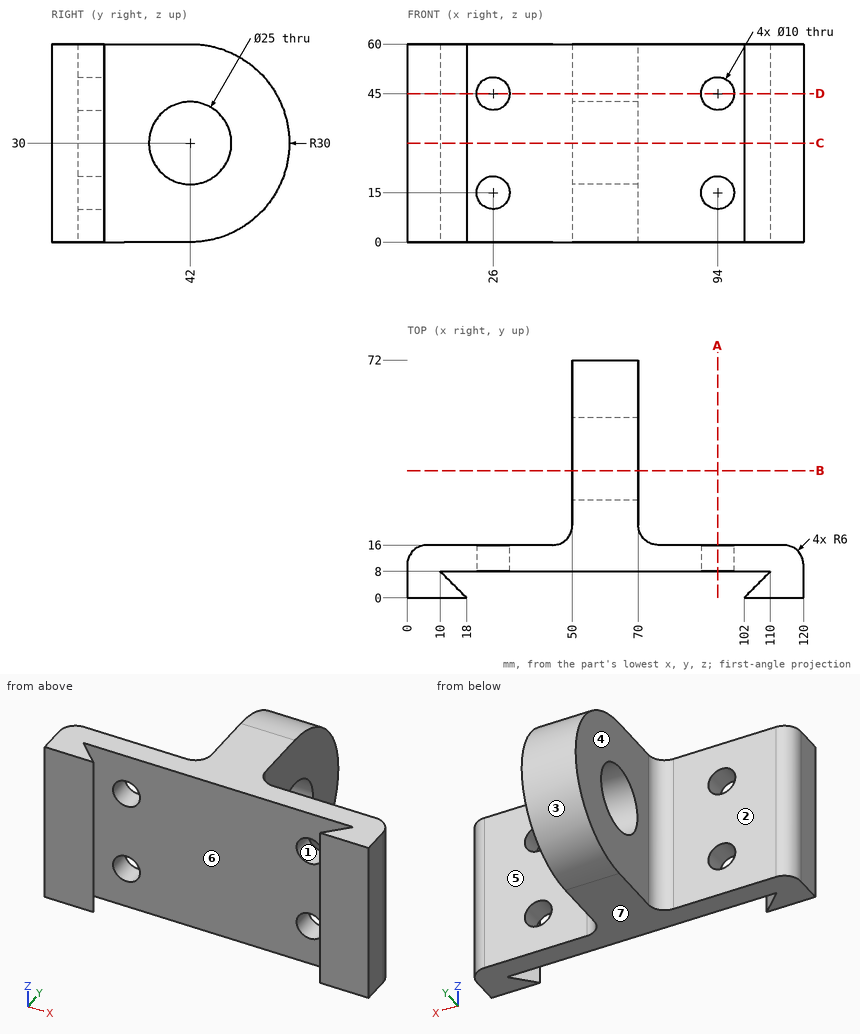
Drawing for the job (mm, zero at the part's lowest x, y, z). A direction names the side the tool comes from. Round coordinates to 2 decimals unless told otherwise and drop trailing zeros. Write each loop counter-clockwise with the first axis right and the second up, starting at its lowest first coordinate (ties: lowest second). Pieces come first, ordered by that corner, then holes. Notation, with made-up numbers: M 32.25,-36.75 L 65.25,-36.75 A8 ccw 65.25,-25.75 Z; hole C -37,3 d2. An arc over 180 degrees is marked long. Put each result on its own line as item: value.
Item 1: Cut at B-B (y = 38.5). List the corners of the cut face in (x, z), and give its area (3 significant figures).
Responses:
outline: M 50,0 L 70,0 L 70,18 L 50,18 Z; M 50,42 L 70,42 L 70,60 L 50,60 Z
area: 720 mm²
Item 2: Cut at C-C (z = 30). List the corners of the cut face in (x, y), and give its area (3 significant figures).
Responses:
outline: M 0,0 L 18,0 L 10,8 L 110,8 L 102,0 L 120,0 L 120,10 A6 ccw 114,16 L 76,16 A6 cw 70,22 L 70,29.5 L 50,29.5 L 50,22 A6 cw 44,16 L 6,16 A6 ccw 0,10 Z; M 50,54.5 L 70,54.5 L 70,72 L 50,72 Z
area: 1,800 mm²
Item 3: Tool access for the marked faces 4, 5, 6 and 7: list every direction of +Z, -Z, +X, -X, +Y, -Y with a clear straight run to the whole face (end or side of a thin tool).
Responses:
face 4: +Z, -Z, -X, +Y
face 5: +Z, -Z, +X, +Y
face 6: +Z, -Z
face 7: -Z, +X, -X, +Y, -Y
Item 4: Probe L1, parallel to Z at x = 26, y = 10; L2, parallel to X at y = 39, z = 10; L3, parallel to Y at x = 31, z = 50. List the from-to ranges inside material, lowest first. Write a range as from..to.
Responses:
L1: 0..10, 20..40, 50..60
L2: 50..70
L3: 8..16
Item 5: Cut at A-A (x = 94). List the corners of the cut face in (y, z).
Responses:
outline: M 8,0 L 16,0 L 16,10 L 8,10 Z; M 8,20 L 16,20 L 16,40 L 8,40 Z; M 8,50 L 16,50 L 16,60 L 8,60 Z
Item 6: Flat gauge pins, fed straight in: P1, Ø16, axis at x = 26, z = 15, coming from the +Y side; P2, Ø18, axis at x = 79.5, z = 16.5, coming from the -Y side; P3, Ø10, axis at x = 62.5, y = 22, coming from the -Z side; P4, Ø25, axis at y = 58.5, z = 16.5, coming from the -X side. Where does each tip first touch, or does it go through?
Responses:
P1: y = 16
P2: y = 8
P3: z = 0
P4: x = 50
Item 7: Cut at D-D (z = 45). List the corners of the cut face in (x, y), and give its area (3 significant figures).
Responses:
outline: M 0,0 L 18,0 L 10,8 L 21,8 L 21,16 L 6,16 A6 ccw 0,10 Z; M 31,8 L 89,8 L 89,16 L 76,16 A6 cw 70,22 L 70,67.98 L 50,67.98 L 50,22 A6 cw 44,16 L 31,16 Z; M 99,8 L 110,8 L 102,0 L 120,0 L 120,10 A6 ccw 114,16 L 99,16 Z
area: 2,060 mm²
Item 8: Mould opens along Z. For the marked faces 1, 2 and 3 say: +Z half, -Z half, draft (parallel to the pull), parting line (faces both ways), or undercut.
Responses:
face 1: undercut
face 2: draft
face 3: parting line
